from build123d import *

# Parameters (mm, degrees)
SKETCH1_W                                           = 100
SKETCH1_H                                           = 50
BOSS_EXTRUDE1_DEPTH                                 = 50
SKETCH2_W                                           = 30
SKETCH2_H                                           = 30
CUT_EXTRUDE1_DEPTH                                  = 115.564392374
CBORE_FOR_M3_HEX_SOCKET_HEAD_CAP_SCREW1_D           = 2
CBORE_FOR_M3_HEX_SOCKET_HEAD_CAP_SCREW1_DEPTH       = 10
CBORE_FOR_M3_HEX_SOCKET_HEAD_CAP_SCREW1_CBORE_D     = 6.5
CBORE_FOR_M3_HEX_SOCKET_HEAD_CAP_SCREW1_CBORE_DEPTH = 3.4
CBORE_FOR_M3_HEX_SOCKET_HEAD_CAP_SCREW2_D           = 2
CBORE_FOR_M3_HEX_SOCKET_HEAD_CAP_SCREW2_CBORE_D     = 6.5
CBORE_FOR_M3_HEX_SOCKET_HEAD_CAP_SCREW2_CBORE_DEPTH = 3.4
M4_TAPPED_HOLE1_D                                   = 3.3
M4_TAPPED_HOLE1_DEPTH                               = 10.1
M4_TAPPED_HOLE1_TIP                                 = 0.991420021
F_4_0_4_DIAMETER_HOLE1_D                            = 4
F_4_0_4_DIAMETER_HOLE1_DEPTH                        = 10
CHAMFER1_SIZE                                       = 2
M8_TAPPED_HOLE1_D                                   = 6.8
M8_TAPPED_HOLE1_DEPTH                               = 19.75
M8_TAPPED_HOLE1_TIP                                 = 2.042926105
M4_TAPPED_HOLE2_D                                   = 3.3
M4_TAPPED_HOLE2_DEPTH                               = 10.1
M4_TAPPED_HOLE2_TIP                                 = 0.991420021
M4_TAPPED_HOLE3_D                                   = 3.3
M4_TAPPED_HOLE3_DEPTH                               = 10.1
M4_TAPPED_HOLE3_TIP                                 = 0.991420021


with BuildPart() as part:
    # Sketch1 → Boss-Extrude1 (new body)
    with BuildSketch(Plane.XY):
        Rectangle(SKETCH1_W, SKETCH1_H)
    extrude(amount=BOSS_EXTRUDE1_DEPTH)

    # Sketch2 → Cut-Extrude1 (cut, through all)
    with BuildSketch(Plane(origin=(50, 0, 0), x_dir=(0, 0, -1), z_dir=(1, 0, 0))):
        with Locations((-25, 0)):
            Rectangle(SKETCH2_W, SKETCH2_H)
    extrude(amount=-CUT_EXTRUDE1_DEPTH, mode=Mode.SUBTRACT)

    # CBORE for M3 Hex Socket Head Cap Screw1
    with Locations(Plane(origin=(0, 0, 0), x_dir=(-1, 0, 0), z_dir=(0, 0, -1))):
        with Locations((-25, 0), (25, 0)):
            CounterBoreHole(CBORE_FOR_M3_HEX_SOCKET_HEAD_CAP_SCREW1_D / 2, CBORE_FOR_M3_HEX_SOCKET_HEAD_CAP_SCREW1_CBORE_D / 2, CBORE_FOR_M3_HEX_SOCKET_HEAD_CAP_SCREW1_CBORE_DEPTH, depth=CBORE_FOR_M3_HEX_SOCKET_HEAD_CAP_SCREW1_DEPTH)

    # CBORE for M3 Hex Socket Head Cap Screw2 (through all)
    with Locations(Plane.XY.offset(50)):
        with Locations((-25, 0), (25, 0)):
            CounterBoreHole(CBORE_FOR_M3_HEX_SOCKET_HEAD_CAP_SCREW2_D / 2, CBORE_FOR_M3_HEX_SOCKET_HEAD_CAP_SCREW2_CBORE_D / 2, CBORE_FOR_M3_HEX_SOCKET_HEAD_CAP_SCREW2_CBORE_DEPTH)

    # M4 Tapped Hole1
    with Locations(Plane.XY.offset(50)):
        with Locations((-35, 0), (35, 0)):
            Hole(M4_TAPPED_HOLE1_D / 2, depth=M4_TAPPED_HOLE1_DEPTH)
            with Locations((0, 0, -(M4_TAPPED_HOLE1_DEPTH + M4_TAPPED_HOLE1_TIP / 2))):  # 118° drill point
                Cone(0, M4_TAPPED_HOLE1_D / 2, M4_TAPPED_HOLE1_TIP, mode=Mode.SUBTRACT)

    # Ø4.0 (4) Diameter Hole1
    with Locations(Plane.XY.offset(50)):
        with Locations((15, 0), (-15, 0)):
            Hole(F_4_0_4_DIAMETER_HOLE1_D / 2, depth=F_4_0_4_DIAMETER_HOLE1_DEPTH)

    # Chamfer1
    chamfer1_edges = [part.edges().sort_by_distance(p)[0] for p in [
        (0, -25, 50),
        (0, -25, 0),
        (0, 25, 0),
        (0, 25, 50),
    ]]
    chamfer(chamfer1_edges, length=CHAMFER1_SIZE)

    # M8 Tapped Hole1
    with Locations(Plane(origin=(0, -25, 0), x_dir=(-1, 0, 0), z_dir=(0, -1, 0))):
        with Locations((0, -25)):
            Hole(M8_TAPPED_HOLE1_D / 2, depth=M8_TAPPED_HOLE1_DEPTH)
            with Locations((0, 0, -(M8_TAPPED_HOLE1_DEPTH + M8_TAPPED_HOLE1_TIP / 2))):  # 118° drill point
                Cone(0, M8_TAPPED_HOLE1_D / 2, M8_TAPPED_HOLE1_TIP, mode=Mode.SUBTRACT)

    # M4 Tapped Hole2
    with Locations(Plane(origin=(0, 0, 3.4), x_dir=(-1, 0, 0), z_dir=(0, 0, -1))):
        with Locations((-25, 0), (25, 0)):
            Hole(M4_TAPPED_HOLE2_D / 2, depth=M4_TAPPED_HOLE2_DEPTH)
            with Locations((0, 0, -(M4_TAPPED_HOLE2_DEPTH + M4_TAPPED_HOLE2_TIP / 2))):  # 118° drill point
                Cone(0, M4_TAPPED_HOLE2_D / 2, M4_TAPPED_HOLE2_TIP, mode=Mode.SUBTRACT)

    # M4 Tapped Hole3
    with Locations(Plane.XY.offset(46.6)):
        with Locations((-25, 0), (25, 0)):
            Hole(M4_TAPPED_HOLE3_D / 2, depth=M4_TAPPED_HOLE3_DEPTH)
            with Locations((0, 0, -(M4_TAPPED_HOLE3_DEPTH + M4_TAPPED_HOLE3_TIP / 2))):  # 118° drill point
                Cone(0, M4_TAPPED_HOLE3_D / 2, M4_TAPPED_HOLE3_TIP, mode=Mode.SUBTRACT)


solid = part.part
Input: part model. Units: mm. Frame: model coordinates. A direction names the side the tool comes from. Coordinates: 2 decimals unless noted, no trailing zeros. Loops run counter-clockwise (first coordinate to the right, second up) from the corner with the lowest first, then second, coordinate; pieces in that order, holes last. Notation, with made-up numbers: (2.5, 77.25) - (23.5, 77.25) arc R28 cw to (23.5, 96.25) - close; hole circle Ø7 at (27, 88.25). An arc over 180 degrees is marked (long way). Answer in a Markdown table with one row per item. Add a question column.
Item 1: Line query: line 1 along Z through (x, y) = (43.5, -5); line 2 along Y through (x, z) = (15, 16.5); line 3 along Y through (x, z) = (-25, 2.5). Output: solid intervals per line, ascending. Write a range as [from, to].
Item 2: Section query C-C on x = 0. Return the cut outline in (y, z), then the cut area to 3 significant figures.
Item 3: Access query for faces 4 (the cylindrical face through (16.6, -1.2, 44.9)), 5 (the flat face through (1, 0, 10)), 6 (the flat face through (-26.4, -1.4, 3.4)). Directions: +Z, -Z, +X, -X, +Y, -Y. A direction counts if a zero-diameter tool reaches every point of the face in a straight line with its end or side. Return the directions, or none.
Item 4: Contact query for flat-ended pins moving along their axis: P1, Ø4, axis at x = 25, y = 0, coming from the +Z side; P2, Ø5.5, axis at x = -25, y = 0, coming from the -Z side. Output: stop coordinate, or through.
Item 5: Section query A-A on y = 14. Return the cut outline in (x, z).
Item 6: Section query D-D on z = 18.5. Return the cut outline in (x, y).
Item 7: Section query B-B on z = 25. Return the cut outline in (x, y).
Item 8: Mould query, pull axis X, two halves, no side actions, for faces 1 (the flat face through (-1, -25, 30)), 2 (the cylindrical face through (-21.753, 0.143, 1.676)), 3 (the flat face through (-50, 0, 41)). Classes: released by +X, released by -X, zero draft, split by the parting line, or undercut.
Recorded:
| question | item | result |
|---|---|---|
| 1 | line 1 | [0, 10], [40, 50] |
| 1 | line 2 | [-25, -15], [15, 25] |
| 1 | line 3 | [-25, -3.25], [3.25, 25] |
| 2 | outline | (-25, 2) - (-23, 0) - (23, 0) - (25, 2) - (25, 48) - (23, 50) - (-23, 50) - (-25, 48) - (-25, 28.4) - (-15, 28.4) - (-15, 40) - (15, 40) - (15, 10) - (-15, 10) - (-15, 21.6) - (-25, 21.6) - close |
| 2 | area | 1,520 mm^2 |
| 3 | face 4 | +Z |
| 3 | face 5 | +X, -X |
| 3 | face 6 | -Z |
| 4 | P1 | z = 46.6 |
| 4 | P2 | z = 3.4 |
| 5 | outline | (-50, 0) - (50, 0) - (50, 10) - (-50, 10) - close; (-50, 40) - (50, 40) - (50, 50) - (-50, 50) - close |
| 6 | outline | (-50, -25) - (50, -25) - (50, -15) - (-50, -15) - close; (-50, 15) - (50, 15) - (50, 25) - (-50, 25) - close |
| 7 | outline | (-50, -25) - (-3.4, -25) - (-3.4, -15) - (-50, -15) - close; (-50, 15) - (50, 15) - (50, 25) - (-50, 25) - close; (3.4, -25) - (50, -25) - (50, -15) - (3.4, -15) - close |
| 8 | face 1 | zero draft |
| 8 | face 2 | undercut |
| 8 | face 3 | released by -X |
